from build123d import *

# Parameters (mm, degrees)
SKETCH_1_W              = 14
SKETCH_1_H              = 14
SKETCH_1_R              = 4
EXTRUDE_1_DEPTH         = 3
HOLE_WIZARD_M3_1_REACH  = 17.937
HOLE_WIZARD_M3_1_BORE_R = 1.25
CHAMFER_2_SIZE          = 2


with BuildPart() as part:
    # 草图1 → 凸台-拉伸1 (new, symmetric)
    with BuildSketch(Plane.XY):
        Rectangle(SKETCH_1_W, SKETCH_1_H)
        Circle(SKETCH_1_R, mode=Mode.SUBTRACT)
    extrude(amount=EXTRUDE_1_DEPTH, both=True)

    # M3 螺纹孔1 bore (on position points) → M3 螺纹孔1 (cut, up to next)
    with BuildSketch(Plane.ZX.offset(7), mode=Mode.PRIVATE) as hole_wizard_m3_1_sk1:
        Circle(HOLE_WIZARD_M3_1_BORE_R)
    hole_wizard_m3_1_tool1 = extrude(hole_wizard_m3_1_sk1.sketch, amount=-HOLE_WIZARD_M3_1_REACH, mode=Mode.PRIVATE) & part.part
    add(hole_wizard_m3_1_tool1.solids().sort_by_distance((0, 7, 0))[0], mode=Mode.SUBTRACT)

    # 倒角2
    chamfer_2_edges = [part.edges().sort_by_distance(p)[0] for p in [
        (7, -7, 0),
        (-7, -7, 0),
        (-7, 7, 0),
        (7, 7, 0),
    ]]
    chamfer(chamfer_2_edges, length=CHAMFER_2_SIZE)


solid = part.part
Design review of the part built by this model. Coordinates are the model's own, in mm. Round coordinates to 2 decimals unless told otherwise and drop trailing zeros. Write each loop counter-clockwise with the first axis right and the second up, starting at its lowest first coordinate (ties: lowest second). Pieces come first, ordered by that corner, then holes. Notation, with made-up numbers: (80.25, 64) -> (88.25, 64) arc R38 ccw to (88.25, 102) -> close; hole circle Ø3 at (-26.75, -29.5). An arc over 180 degrees is marked (long way). One line per item, written item: value. Start each with the question number.
Q1. The part is to be moulded in two halves that separate along X. For faces 1 (the face through (7, 0, 0)), 2 (the face through (-1.22, 5.42, -0.27)), 3 (the face through (-0.867, -3.905, -0.042)), 4 (the face through (-6, -6, 0)), say which applies: pulls with the +X half, pulls with the -X half, needs draft (parallel to the pull), parting line crosses it, or undercut.
Q2. Add section B-B (x = 3). Give the boundary of the cut face in (y, z), then the cut area to 3 significant figures.
Q3. Add section A-A (y = 0). Give the boundary of the cut face in (x, z).
Q4. Add section C-C (z = 2.25). Give the boundary of the cut face in (x, y).
Q5. To check wall thickness, follow probe 1 along Y at (x, z) = (0, -1.5); probe 2 along Z at (x, y) = (0, 5.9); probe 3 along X at (y, z) = (-0.5, 2). State the ranges of each line that lie inside material, in increasing order.
Q6. Add section D-D (z = 0). Give the boundary of the cut face in (x, y), then the cut area to 3 significant figures.
Response:
1. face 1: pulls with the +X half
1. face 2: undercut
1. face 3: undercut
1. face 4: pulls with the -X half
2. outline: (-7, -3) -> (-2.65, -3) -> (-2.65, 3) -> (-7, 3) -> close; (2.65, -3) -> (7, -3) -> (7, 3) -> (2.65, 3) -> close
2. area: 52.3 mm^2
3. outline: (-7, -3) -> (-4, -3) -> (-4, 3) -> (-7, 3) -> close; (4, -3) -> (7, -3) -> (7, 3) -> (4, 3) -> close
4. outline: (-7, -5) -> (-5, -7) -> (5, -7) -> (7, -5) -> (7, 5) -> (5, 7) -> (-5, 7) -> (-7, 5) -> close; hole circle Ø8 at (0, 0)
5. probe 1: y = -7 to -4, 4 to 7
5. probe 2: z = -3 to -1.25, 1.25 to 3
5. probe 3: x = -7 to -3.97, 3.97 to 7
6. outline: (-7, -5) -> (-5, -7) -> (5, -7) -> (7, -5) -> (7, 5) -> (5, 7) -> (1.25, 7) -> (1.25, 3.8) arc R4 cw (long way) to (-1.25, 3.8) -> (-1.25, 7) -> (-5, 7) -> (-7, 5) -> close
6. area: 130 mm^2
